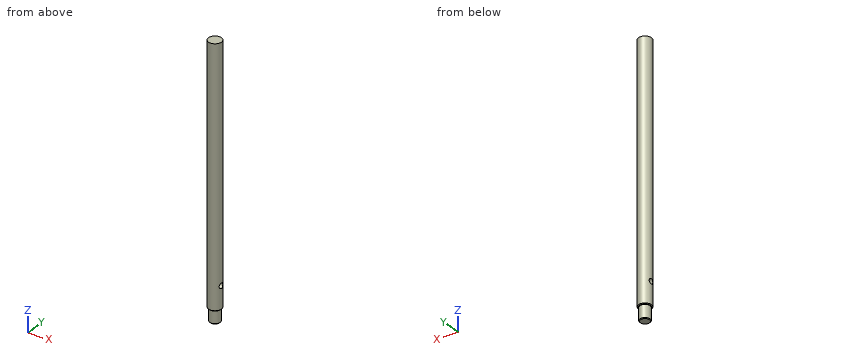
from build123d import *

# Parameters (mm, degrees)
SKETCH2_W               = 150
SKETCH2_H               = 10
CUT_EXTRUDE1_DEPTH      = 10
CUT_EXTRUDE1_DEPTH_BACK = 10
SKETCH5_R               = 4
SKETCH6_R               = 10
BOSS_EXTRUDE1_DEPTH     = 20
SKETCH7_R               = 8
BOSS_EXTRUDE2_DEPTH     = 20
CHAMFER1_SIZE           = 1
BOSS_EXTRUDE4_START     = 220
SKETCH8_R               = 10
BOSS_EXTRUDE4_DEPTH     = 220


with BuildPart() as part:
    # Sketch2 → Revolve4 (revolve)
    with BuildSketch(Plane(origin=(0, 0, 0), x_dir=(0, 0, -1), z_dir=(1, 0, 0)), mode=Mode.PRIVATE) as revolve4_sk:
        with Locations((75, 5)):
            Rectangle(SKETCH2_W, SKETCH2_H)
    revolve(revolve4_sk.sketch.rotate(Axis((0, 0, 0), (0, 0, -1)), 90), axis=Axis((0, 0, 0), (0, 0, -1)))

    # Sketch5 → Cut-Extrude1 (cut, two sides: drawn at the far end of the back side and taken through both)
    with BuildSketch(Plane(origin=(0, 0, 0), x_dir=(0, 0, -1), z_dir=(1, 0, 0)).offset(-CUT_EXTRUDE1_DEPTH_BACK)):
        with Locations(Location((135, 0, 0), (0, 0, 180))):
            Circle(SKETCH5_R)
    extrude(amount=CUT_EXTRUDE1_DEPTH + CUT_EXTRUDE1_DEPTH_BACK, mode=Mode.SUBTRACT)

    # Sketch6 → Boss-Extrude1 (add)
    with BuildSketch(Plane(origin=(0, 0, -150), x_dir=(-1, 0, 0), z_dir=(0, 0, -1))):
        with Locations(Location((0, 0, 0), (0, 0, 180))):
            Circle(SKETCH6_R)
    extrude(amount=BOSS_EXTRUDE1_DEPTH)

    # Sketch7 → Boss-Extrude2 (add)
    with BuildSketch(Plane(origin=(0, 0, -170), x_dir=(-1, 0, 0), z_dir=(0, 0, -1))):
        Circle(SKETCH7_R)
    extrude(amount=BOSS_EXTRUDE2_DEPTH)

    # Chamfer1
    chamfer1_edges = [part.edges().sort_by_distance(p)[0] for p in [
        (-10, 0, -170),
        (8, 0, -190),
    ]]
    chamfer(chamfer1_edges, length=CHAMFER1_SIZE)

    # Sketch8 → Boss-Extrude4 (add)
    with BuildSketch(Plane.XY.offset(BOSS_EXTRUDE4_START)):
        Circle(SKETCH8_R)
    extrude(amount=-BOSS_EXTRUDE4_DEPTH)


solid = part.part
Here's how the part is built. I have some questions about the finished solid (model axes, mm). Coordinates: 2 decimals unless noted, no trailing zeros. Order: outer loops, then holes, each group sorted by start corner. A loop starts at its lowest first (then second) coordinate and runs counter-clockwise, first axis right, second up.
Item 1: If we section it at D-D on z = -80: List the corners of the cut face in (x, y) for me.
Result sheet:
outline: circle Ø20 at (0, 0)
Item 2: If we section it at C-C on z = -135: List the corners of the cut face in (x, y) for me, plus the area to 3 significant figures.
Result sheet:
outline: (-9.17, -4) arc R10 ccw to (9.17, -4) - close; (-9.17, 4) - (9.17, 4) arc R10 ccw to start
area: 159 mm2
Item 3: If we section it at A-A on y = 0: List the corners of the cut face in (x, z) for me.
Result sheet:
outline: (-10, -169) - (-9, -170) - (-8, -170) - (-8, -189) - (-7, -190) - (7, -190) - (8, -189) - (8, -170) - (9, -170) - (10, -169) - (10, -139) - (-10, -139) - close; (-10, -131) - (10, -131) - (10, 220) - (-10, 220) - close
Item 4: For P1, Ø4, axis at x = 1.5, z = 2.5, coming from the -Y side; P2, Ø5, axis at x = -5, z = 108, coming from the -Y side; P3, Ø1.5, axis at x = -8, z = -76.5, coming from the -Y side; P4, Ø3, axis at x = 3.5, z = 133, coming from the -Y side, each with a flat end and sliding along its axis, tell me the tip position at first contact or that it passes through.
Result sheet:
P1: stops at y = -10
P2: stops at y = -9.68
P3: stops at y = -6.89
P4: stops at y = -9.8
Item 5: I need wall thicknesses on line 1 (Y direction, x = -6, z = -55.5); line 2 (Y direction, x = 1.25, z = -143); line 3 (Y direction, x = -5.5, z = -135). Which ranges of each line are inside material? Lowest first, please.
Result sheet:
line 1: y = -8 to 8
line 2: y = -9.92 to 9.92
line 3: y = -8.35 to -4, 4 to 8.35
Item 6: If we section it at B-B on x = 0: List the corners of the cut face in (y, z) for me, plus the area to 3 significant figures.
Result sheet:
outline: (-10, -169) - (-9, -170) - (-8, -170) - (-8, -189) - (-7, -190) - (7, -190) - (8, -189) - (8, -170) - (9, -170) - (10, -169) - (10, 220) - (-10, 220) - close; hole circle Ø8 at (0, -135)
area: 8,070 mm2
